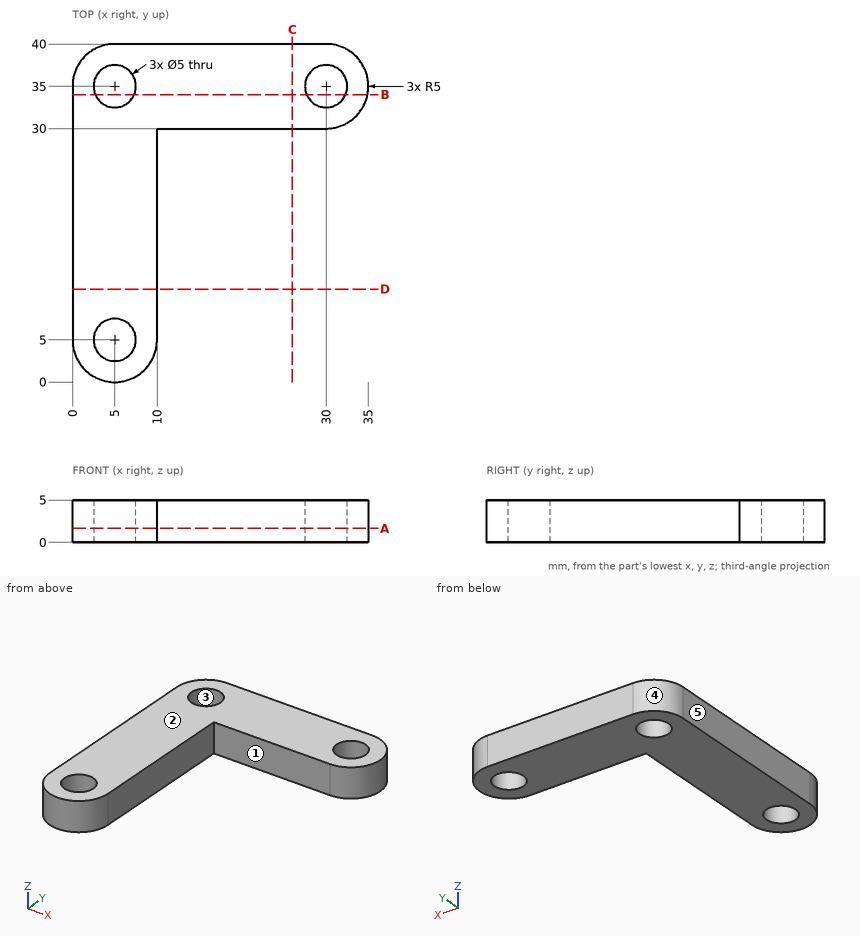
Check sheet for the drawn part. Datum: minimum x, y, z corner. Units: mm. A direction names the side the tool comes from. Round coordinates to 2 decimals unless told otherwise and drop trailing zeros. Loops run counter-clockwise (first coordinate to the right, second up) from the corner with the lowest first, then second, coordinate; pieces in that order, holes last.
Item 1: Thickness scan on line 1 (Y direction, x = 5, z = 3.7); line 2 (Y direction, x = 30, z = 2.3); line 3 (Y direction, x = 20.5, z = 0.3). Record the ranges inside material, lowest first.
Item 2: Access from +Z, -Z, +X, -X, +Y, -Y to the whole of each face (thin tool, end or side, straight path). Record for the marked faces 1 and 2.
Item 3: Cross-section at C-C on x = 26. Record the boundary of the cut face in (y, z).
Item 4: Cross-section at B-B on y = 34. Record the boundary of the cut face in (x, z), then the cut area to 3 significant figures.
Item 5: Gauge pin test, flat ends, axial feed: pin 1 (4 mm diameter, centred on x = 5, y = 35, fed in from -Z); pin 2 (1.5 mm diameter, centred on y = 9.5, z = 2, fed in from +X). Record the tip position at first contact, or that the pin passes through.
Item 6: Cross-section at A-A on z = 1.65. Record the boundary of the cut face in (x, y).
Item 7: Mould release check, pull along Y, two halves, no side actions. Record for the marked faces 3, 4 and 5: pulls with the +Y half, pulls with the -Y half, needs draft (parallel to the pull), parting line crosses it, or undercut.
Item 8: Cross-section at D-D on y = 11. Record the boundary of the cut face in (x, z).
Answer sheet:
1. line 1: y = 0 to 2.5, 7.5 to 32.5, 37.5 to 40
1. line 2: y = 30 to 32.5, 37.5 to 40
1. line 3: y = 30 to 40
2. face 1: +Z, -Z, +X, -Y
2. face 2: +Z, +X, -X, +Y, -Y
3. outline: (30, 0) - (40, 0) - (40, 5) - (30, 5) - close
4. outline: (0, 0) - (2.71, 0) - (2.71, 5) - (0, 5) - close; (7.29, 0) - (27.71, 0) - (27.71, 5) - (7.29, 5) - close; (32.29, 0) - (34.9, 0) - (34.9, 5) - (32.29, 5) - close
4. area: 129 mm2
5. pin 1: passes through
5. pin 2: stops at x = 10
6. outline: (0, 5) arc R5 ccw to (10, 5) - (10, 30) - (30, 30) arc R5 ccw to (30, 40) - (5, 40) arc R5 ccw to (0, 35) - close; hole circle Ø5 at (5, 5); hole circle Ø5 at (5, 35); hole circle Ø5 at (30, 35)
7. face 3: undercut
7. face 4: pulls with the +Y half
7. face 5: needs draft
8. outline: (0, 0) - (10, 0) - (10, 5) - (0, 5) - close
